Verification items for the finished model (mm, model axes). Face numbers are marked on the shaded views. A direction names the side the tool comes from. Round coordinates to 2 decimals unless told otherwise and drop trailing zeros. Write each loop counter-clockwise with the first axis right and the second up, starting at its lowest first coordinate (ties: lowest second). Pieces come first, ordered by that corner, then holes. Notation, with made-up numbers: (-18, 3.5) -> (-5, 3.5) arc R35 cw to (-5, 37.5) -> close; hole circle Ø6 at (53, -13). An arc over 180 degrees is marked (long way). Answer as a JSON object with one key per item and string values. Group by question number.
(1) Sectioned sample at B-B on y = -39. Record the cut outline in (x, z), and give its area (3 significant figures).
(2) Set-up check for the marked faces 1, 2, 3 and 4: record each of +Z, -Z, +X, -X, +Y, -Y from which the full face is reachable in a straight line by a thin tool's end or side.
(3) Sectioned sample at A-A on z = -1.5. Record the cut outline in (x, y).
(4) Sectioned sample at C-C on y = -10.5. Record the cut outline in (x, z).
(5) Gauge pin test, flat ends, axial feed: pin 1 Ø4 at (x, z) = (19.5, -3) entering from -Y; pin 2 Ø1 at (y, z) = (-41, -1) entering from +X; pin 3 Ø4 at (y, z) = (48, -1) entering from -X. Record the tip position at first contact, or that the pin passes through.
(6) Scan lines: L1, parallel to X at y = -33.5, z = 0.5; L2, parallel to X at y = -2.5, z = -3.5; L3, parallel to Y at x = -23, z = -2.5. Record each from-to range of solid material in increasing order. Write a range as from..to.
```python
from build123d import *

# Parameters (mm, degrees)
SKETCH_1_R      = 32.5
EXTRUDE_1_DEPTH = 4
SKETCH_2_W      = 44
SKETCH_2_H      = 130
EXTRUDE_2_DEPTH = 8
CHAMFER_1_SIZE  = 5


with BuildPart() as part:
    # 草图1 → 凸台-拉伸1 (new, symmetric)
    with BuildSketch(Plane.XY):
        Circle(SKETCH_1_R)
    extrude(amount=EXTRUDE_1_DEPTH, both=True)

    # 草图2 → 凸台-拉伸2 (add)
    with BuildSketch(Plane.XY.offset(4)):
        Rectangle(SKETCH_2_W, SKETCH_2_H)
    extrude(amount=-EXTRUDE_2_DEPTH)

    # 倒角1
    chamfer_1_edges = [part.edges().sort_by_distance(p)[0] for p in [
        (22, 65, 0),
        (-22, -65, 0),
        (22, -65, 0),
        (-22, 65, 0),
    ]]
    chamfer(chamfer_1_edges, length=CHAMFER_1_SIZE)


solid = part.part
```
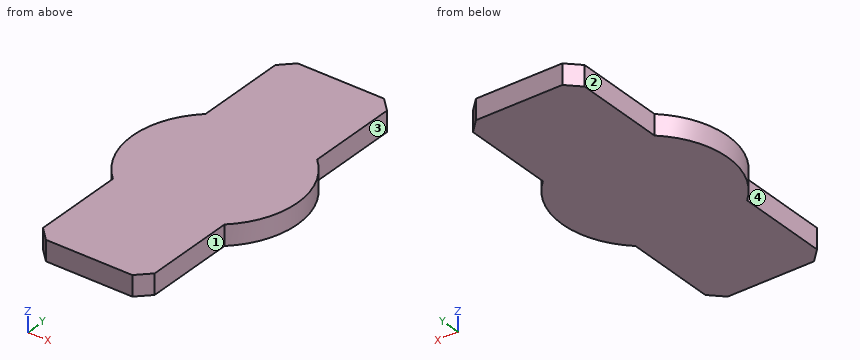
Computed values:
{
 "1": {"outline": "(-22, -4) -> (22, -4) -> (22, 4) -> (-22, 4) -> close", "area": "352 mm2"},
 "2": {"face 1": "+Z, -Z, +X, -Y", "face 2": "+Z, -Z, -X, +Y", "face 3": "+Z, -Z, +X, +Y", "face 4": "+Z, -Z, -X, -Y"},
 "3": {"outline": "(-22, -60) -> (-17, -65) -> (17, -65) -> (22, -60) -> (22, -23.92) arc R32.5 ccw to (22, 23.92) -> (22, 60) -> (17, 65) -> (-17, 65) -> (-22, 60) -> (-22, 23.92) arc R32.5 ccw to (-22, -23.92) -> close"},
 "4": {"outline": "(-30.76, -4) -> (30.76, -4) -> (30.76, 4) -> (-30.76, 4) -> close"},
 "5": {"pin 1": "y = -64.5", "pin 2": "x = 22", "pin 3": "x = -22"},
 "6": {"L1": "-22..22", "L2": "-32.4..32.4", "L3": "-22.96..22.96"}
}
